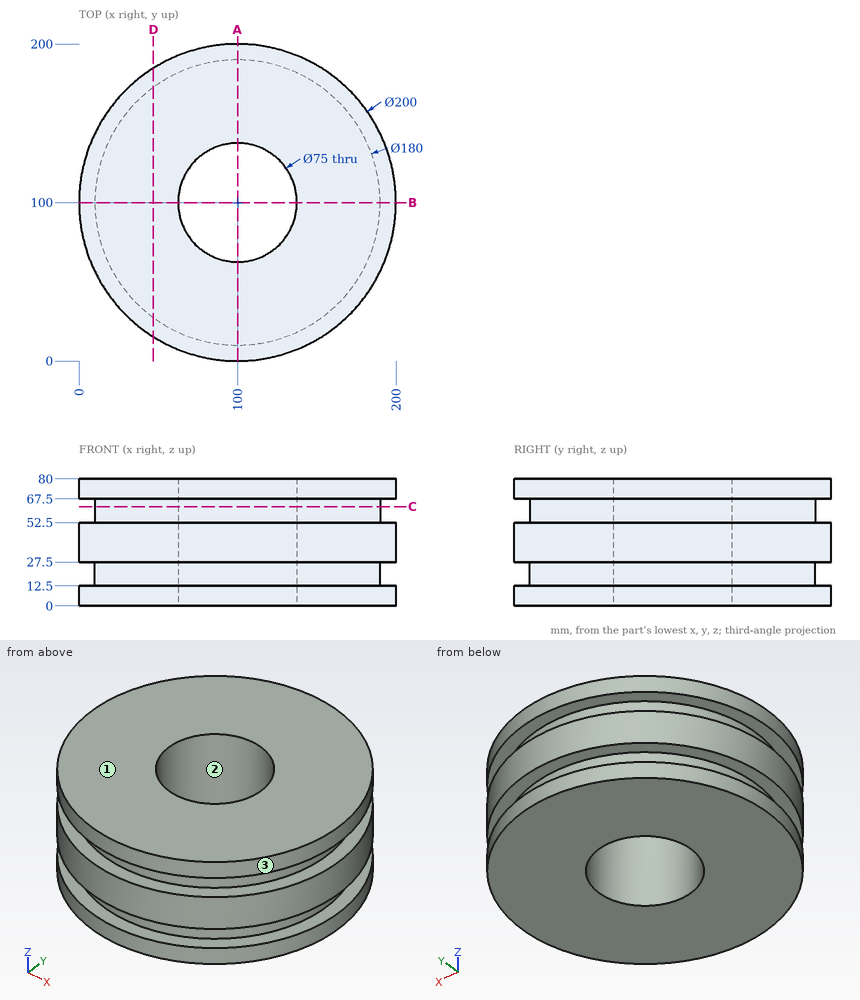
Input: dimensioned drawing with shaded views. Units: mm. Origin: part minimum x, y, z. Coordinates: 2 decimals unless noted, no trailing zeros. Order: outer loops, then holes, each group sorted by start corner. A loop starts at its lowest first (then second) coordinate and runs counter-clockwise, first axis right, second up.
1. Cut plane A-A, the plane x = 100. Return loops of the section in (y, z), plus the area to 3 significant figures.
Checked values:
outline: (0, 0) - (62.5, 0) - (62.5, 80) - (0, 80) - (0, 67.5) - (10, 67.5) - (10, 52.5) - (0, 52.5) - (0, 27.5) - (10, 27.5) - (10, 12.5) - (0, 12.5) - close; (137.5, 0) - (200, 0) - (200, 12.5) - (190, 12.5) - (190, 27.5) - (200, 27.5) - (200, 52.5) - (190, 52.5) - (190, 67.5) - (200, 67.5) - (200, 80) - (137.5, 80) - close
area: 9,400 mm2
2. Cut plane C-C, the plane z = 62.5. Return loops of the section in (x, y), plus the area to 3 significant figures.
Checked values:
outline: circle Ø180 at (100, 100); hole circle Ø75 at (100, 100)
area: 21,000 mm2
3. Cut plane D-D, the plane x = 47. Return loops of the section in (y, z), plus the area to 3 significant figures.
Checked values:
outline: (15.2, 0) - (184.8, 0) - (184.8, 12.5) - (172.74, 12.5) - (172.74, 27.5) - (184.8, 27.5) - (184.8, 52.5) - (172.74, 52.5) - (172.74, 67.5) - (184.8, 67.5) - (184.8, 80) - (15.2, 80) - (15.2, 67.5) - (27.26, 67.5) - (27.26, 52.5) - (15.2, 52.5) - (15.2, 27.5) - (27.26, 27.5) - (27.26, 12.5) - (15.2, 12.5) - close
area: 12,800 mm2
4. Contact query for flat-ended pins moving along their axis: P1, Ø2, axis at x = 128, z = 30.5, coming from the -Y side; P2, Ø2, axis at y = 124, z = 35.5, coming from the +X side; P3, Ø10, axis at x = 142, y = 111, coming from the -Z side; P4, Ø4, axis at y = 55.5, z = 61.5, coming from the +X side. Output: stop coordinate, or through.
Checked values:
P1: stops at y = 3.71
P2: stops at x = 197.32
P3: stops at z = 0
P4: stops at x = 179.33
5. Draft query along Y for the marked faces 1, 2 and 3. Return one class per face: +Y half, -Y half, draft (parallel to the pull), parting line (faces both ways), or undercut.
Checked values:
face 1: draft
face 2: undercut
face 3: parting line
6. Ray query, line 1 along Z through (x, y) = (12, 130); line 2 along Y through (x, z) = (100, 43); line 3 along X through (y, z) = (98, 46). Return the intervals inside material, ascending.
Checked values:
line 1: z = 0 to 12.5, 27.5 to 52.5, 67.5 to 80
line 2: y = 0 to 62.5, 137.5 to 200
line 3: x = 0.02 to 62.55, 137.45 to 199.98
